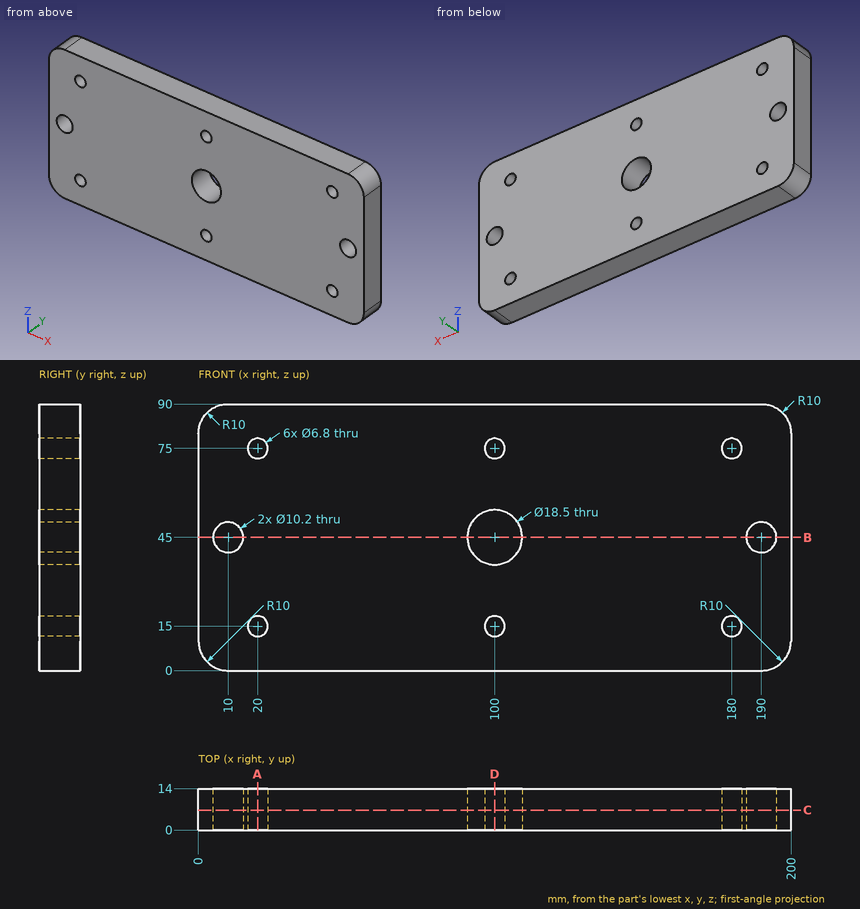
Verification items for this drawing (mm, ordinates from the low corner). Coordinates: 2 decimals unless noted, no trailing zeros. Loops run counter-clockwise (first coordinate to the right, second up) from the corner with the lowest first, then second, coordinate; pieces in that order, holes last. Notation, with made-up numbers: (55, 84) -> (61, 84) arc R11 cw to (61, 98) -> close; hole circle Ø6 at (85.5, -2.75). An arc over 180 degrees is marked (long way). Answer in a Markdown table with one row per item. Add a question column.
1. Section check B-B, the plane z = 45. Enter the section's corners in (x, y), then the cut area to 3 significant figures.
2. Section check A-A, the plane x = 20. Enter the section's corners in (y, z).
3. Material ranges on probe 1 along X at (y, z) = (9.5, 15); probe 2 along Z at (x, y) = (100, 4); probe 3 along Z at (x, y) = (20, 4.25), recorded low to high. Write a range as [from, to].
4. Section check D-D, the plane x = 100. Enter the section's corners in (y, z), then the cut area to 3 significant figures.
5. Section check C-C, the plane y = 6.75. Give the number of separate pieces and of enclosed holes in the cut face, then the cut area to 3 significant figures.
Derived:
| question | item | result |
|---|---|---|
| 1 | outline | (0, 0) -> (4.9, 0) -> (4.9, 14) -> (0, 14) -> close; (15.1, 0) -> (90.75, 0) -> (90.75, 14) -> (15.1, 14) -> close; (109.25, 0) -> (184.9, 0) -> (184.9, 14) -> (109.25, 14) -> close; (195.1, 0) -> (200, 0) -> (200, 14) -> (195.1, 14) -> close |
| 1 | area | 2,260 mm² |
| 2 | outline | (0, 0) -> (14, 0) -> (14, 11.6) -> (0, 11.6) -> close; (0, 18.4) -> (14, 18.4) -> (14, 71.6) -> (0, 71.6) -> close; (0, 78.4) -> (14, 78.4) -> (14, 90) -> (0, 90) -> close |
| 3 | probe 1 | x = [0, 16.6], [23.4, 96.6], [103.4, 176.6], [183.4, 200] |
| 3 | probe 2 | z = [0, 11.6], [18.4, 35.75], [54.25, 71.6], [78.4, 90] |
| 3 | probe 3 | z = [0, 11.6], [18.4, 71.6], [78.4, 90] |
| 4 | outline | (0, 0) -> (14, 0) -> (14, 11.6) -> (0, 11.6) -> close; (0, 18.4) -> (14, 18.4) -> (14, 35.75) -> (0, 35.75) -> close; (0, 54.25) -> (14, 54.25) -> (14, 71.6) -> (0, 71.6) -> close; (0, 78.4) -> (14, 78.4) -> (14, 90) -> (0, 90) -> close |
| 4 | area | 811 mm² |
| 5 | separate pieces | 1 |
| 5 | enclosed holes | 9 |
| 5 | area | 17,300 mm² |
